Study the drawing (mm; zero at the part's minimum x, y, z) and answer. Give positions to 0.01 mm unless a question says otherwise; leave off trailing zeros. Order: outer loops, then holes, each group sorted by start corner. A loop starts at its lowest first (then second) coordinate and runs counter-clockwise, first axis right, second up. Notation, with made-up numbers: (65, -14.5) -> (98, -14.5) arc R11 cw to (98, -6.5) -> close; hole circle Ø7 at (6.5, -18). An arc over 180 degrees is marked (long way). Use a Markdown table: item, result. Add a question column.
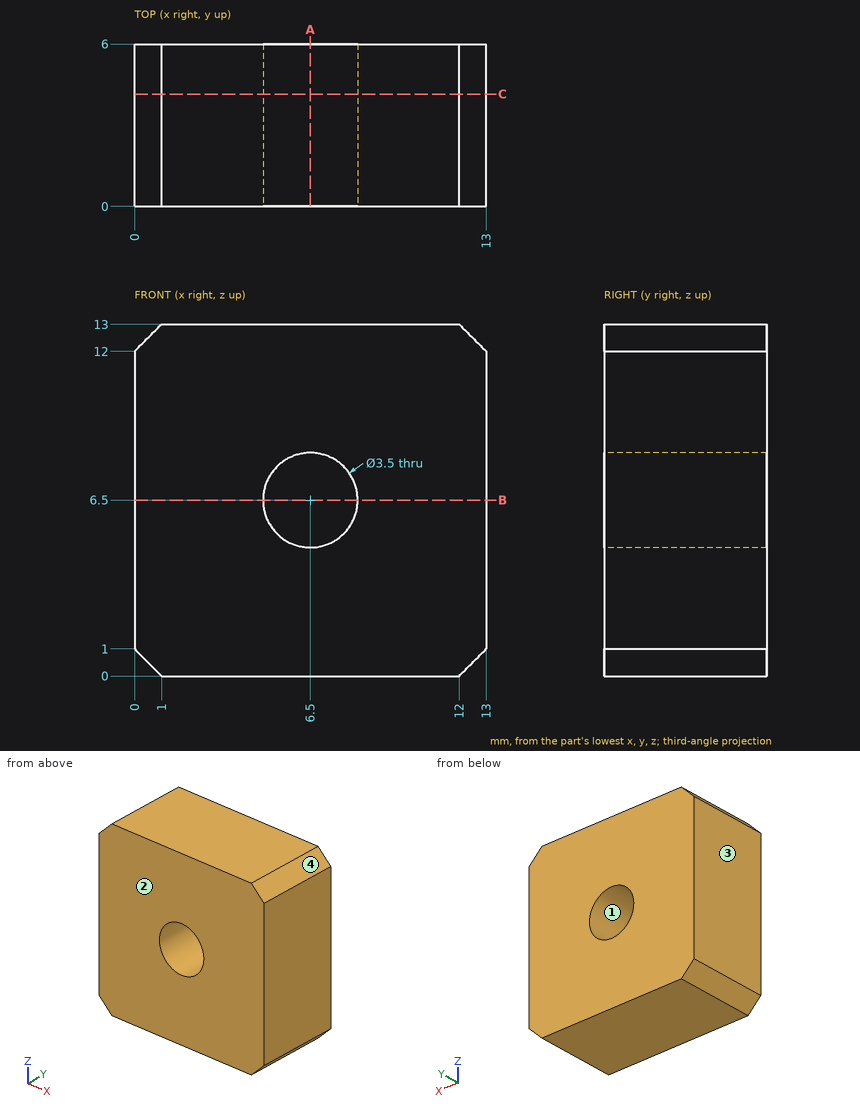
1) A flat-ended cylindrical pin translates along its axis: pin 1 (4.5 mm diameter, centred on x = 6.5, z = 6.5, fed in from +Y). Find the tip coordinate at first contact, or state that the pin passes through.
2) The part is cut by section C-C, the plane y = 4.15. Determine the outline of the cut face in (x, z), then the cut area to 3 significant figures.
3) Straight lines are drawn through the part: line 1 (X direction, y = 3.8, z = 6.5); line 2 (Z direction, x = 5.5, y = 2.4). For each, find the intervals that lie inside material, in ascending order.
4) Determine the mould class of the marked faces 1, 2, 3 and 4 for opening direction X: released by +X, released by -X, zero draft, split by the parting line, or undercut.
5) The part is cut by section B-B, the plane z = 6.5. Determine the outline of the cut face in (x, y).
6) The part is cut by section A-A, the plane x = 6.5. Determine the outline of the cut face in (y, z), then the cut area to 3 significant figures.
A:
| question | item | result |
|---|---|---|
| 1 | pin 1 | y = 6 |
| 2 | outline | (0, 1) -> (1, 0) -> (12, 0) -> (13, 1) -> (13, 12) -> (12, 13) -> (1, 13) -> (0, 12) -> close; hole circle Ø3.5 at (6.5, 6.5) |
| 2 | area | 157 mm^2 |
| 3 | line 1 | 0 to 4.75, 8.25 to 13 |
| 3 | line 2 | 0 to 5.06, 7.94 to 13 |
| 4 | face 1 | undercut |
| 4 | face 2 | zero draft |
| 4 | face 3 | released by -X |
| 4 | face 4 | released by +X |
| 5 | outline | (0, 0) -> (4.75, 0) -> (4.75, 6) -> (0, 6) -> close; (8.25, 0) -> (13, 0) -> (13, 6) -> (8.25, 6) -> close |
| 6 | outline | (0, 0) -> (6, 0) -> (6, 4.75) -> (0, 4.75) -> close; (0, 8.25) -> (6, 8.25) -> (6, 13) -> (0, 13) -> close |
| 6 | area | 57.0 mm^2 |
